Source: CAD feature listing. Evaluate the final solid. Frame: model axes, mm. A direction names the side the tool comes from. Give positions to 0.01 mm unless a question says otherwise; leave off trailing zeros. Loops run counter-clockwise (first coordinate to the right, second up) from the corner with the lowest first, then second, coordinate; pieces in that order, holes last. Notation, with made-up numbers: M 41.5,-16 L 84.5,-16 A24 cw 84.5,10 Z; hole C 31,-7.75 d2. An arc over 180 degrees is marked long. Put each result on its own line as item: value.
from build123d import *

# Parameters (mm, degrees)
SKETCH1_W               = 720
SKETCH1_H               = 365
BOSS_EXTRUDE1_DEPTH     = 20
CUT_EXTRUDE1_DEPTH      = 405.111680108
CUT_EXTRUDE1_DEPTH_BACK = 405.111680108
SKETCH2_R               = 20
CHAMFER1_SIZE           = 20
CHAMFER2_SIZE           = 20
CUT_EXTRUDE2_DEPTH      = 405.111680108
CUT_EXTRUDE2_DEPTH_BACK = 405.111680108
SKETCH4_W               = 480
SKETCH4_H               = 370


with BuildPart() as part:
    # Sketch1 → Boss-Extrude1 (new body)
    with BuildSketch(Plane.XY):
        Rectangle(SKETCH1_W, SKETCH1_H)
    extrude(amount=BOSS_EXTRUDE1_DEPTH)

    # Sketch2 → Cut-Extrude1 (cut, two sides: drawn at the far end of the back side and taken through both)
    with BuildSketch(Plane.XY.offset(20).offset(-CUT_EXTRUDE1_DEPTH_BACK)):
        with Locations((-310, 102.5)):
            Circle(SKETCH2_R)
        with Locations((310, 102.5)):
            Circle(SKETCH2_R)
    extrude(amount=CUT_EXTRUDE1_DEPTH + CUT_EXTRUDE1_DEPTH_BACK, mode=Mode.SUBTRACT)

    # Chamfer1
    chamfer1_edges = [part.edges().sort_by_distance(p)[0] for p in [
        (-360, 182.5, 10),
        (360, 182.5, 10),
    ]]
    chamfer(chamfer1_edges, length=CHAMFER1_SIZE)

    # Chamfer2
    chamfer2_edges = [part.edges().sort_by_distance(p)[0] for p in [
        (360, -182.5, 10),
        (-360, -182.5, 10),
    ]]
    chamfer(chamfer2_edges, length=CHAMFER2_SIZE)

    # Sketch4 → Cut-Extrude2 (cut, two sides: drawn at the far end of the back side and taken through both)
    with BuildSketch(Plane.XY.offset(20).offset(-CUT_EXTRUDE2_DEPTH_BACK)):
        with Locations((0, -182.5)):
            Rectangle(SKETCH4_W, SKETCH4_H)
    extrude(amount=CUT_EXTRUDE2_DEPTH + CUT_EXTRUDE2_DEPTH_BACK, mode=Mode.SUBTRACT)


solid = part.part
1. Material intervals for line 1 (X direction, y = 102.5, z = 14); line 2 (X direction, y = -60.5, z = 15.5); line 3 (Y direction, x = 310, z = 5.75), sorted ascending. Write a range as from..to.
Found:
line 1: -360..-330, -290..290, 330..360
line 2: -360..-240, 240..360
line 3: -182.5..82.5, 122.5..182.5
2. Section query B-B (y = -28.5). Output: boundary loops of the cut face in (x, z).
Found:
outline: M -360,0 L -240,0 L -240,20 L -360,20 Z; M 240,0 L 360,0 L 360,20 L 240,20 Z
3. Draft query along X for faces 1 (the flat face through (-5, 43, 20)), 2 (the cylindrical face through (328.475, 94.84, 9.86)), 3 (the flat face through (360, -2, 10)). Return one class per face: pulls with the +X half, pulls with the -X half, needs draft (parallel to the pull), parting line crosses it, or undercut.
Found:
face 1: needs draft
face 2: undercut
face 3: pulls with the +X half
4. Contact query for a flat-ended pin moving along its axis: P1, Ø10, axis at x = -179, z = 11.5, coming from the -Y side. Output: stop coordinate, or through.
Found:
P1: y = 2.5
5. Section query A-A (x = 310). Output: boundary loops of the cut face in (y, z), plus the area to 3 significant figures.
Found:
outline: M -182.5,0 L 82.5,0 L 82.5,20 L -182.5,20 Z; M 122.5,0 L 182.5,0 L 182.5,20 L 122.5,20 Z
area: 6,500 mm^2
6. Section query C-C (y = 102.5). Output: boundary loops of the cut face in (x, z), plus the area to 3 significant figures.
Found:
outline: M -360,0 L -330,0 L -330,20 L -360,20 Z; M -290,0 L 290,0 L 290,20 L -290,20 Z; M 330,0 L 360,0 L 360,20 L 330,20 Z
area: 12,800 mm^2
7. Access query for faces 4 (the flat face through (240, -91, 10)), 5 (the flat face through (-5, 182.5, 10)). Directions: +Z, -Z, +X, -X, +Y, -Y. A direction counts if a zero-diameter tool reaches every point of the face in a straight line with its end or side. Return the directions, or none.
Found:
face 4: +Z, -Z, -Y
face 5: +Z, -Z, +X, -X, +Y
8. Section query D-D (z = 5.5). Output: boundary loops of the cut face in (x, y).
Found:
outline: M -360,-162.5 L -340,-182.5 L -240,-182.5 L -240,2.5 L 240,2.5 L 240,-182.5 L 340,-182.5 L 360,-162.5 L 360,162.5 L 340,182.5 L -340,182.5 L -360,162.5 Z; hole C -310,102.5 d40; hole C 310,102.5 d40
